```python
from build123d import *

# Parameters (mm, degrees)
BOSS_EXTRUDE1_DEPTH = 1440
SKETCH2_R           = 8.5
CUT_EXTRUDE1_DEPTH  = 1440


with BuildPart() as part:
    # Sketch1 → Boss-Extrude1 (new body)
    with BuildSketch(Plane.XY):
        with BuildLine():
            Line((0, 0), (-50, 0))
            Line((-50, 0), (-50, -100))
            Line((-50, -100), (0, -100))
            Line((0, -100), (0, -98.925311188))
            ThreePointArc((0, -98.925311188), (-1.103806889, -95.973045557), (-3.873721046, -94.469104878))
            Line((-3.873721046, -94.469104878), (-36.682971358, -89.858065454))
            ThreePointArc((-36.682971358, -89.858065454), (-41.915031432, -87.017288616), (-44, -81.440786869))
            Line((-44, -81.440786869), (-44, -18.559213131))
            ThreePointArc((-44, -18.559213131), (-41.915031432, -12.982711384), (-36.682971358, -10.141934546))
            Line((-36.682971358, -10.141934546), (-3.873721046, -5.530895122))
            ThreePointArc((-3.873721046, -5.530895122), (-1.103806889, -4.026954443), (0, -1.074688812))
            Line((0, -1.074688812), (0, 0))
        make_face()
    extrude(amount=BOSS_EXTRUDE1_DEPTH)

    # Sketch2 → Cut-Extrude1 (cut)
    with BuildSketch(Plane.ZY.offset(50)):
        with Locations(Location((73.2, -38, 0), (0, 0, 270))):
            Circle(SKETCH2_R)
        with Locations(Location((234.9, -38, 0), (0, 0, 270))):
            Circle(SKETCH2_R)
        with Locations(Location((396.6, -38, 0), (0, 0, 270))):
            Circle(SKETCH2_R)
        with Locations(Location((558.3, -38, 0), (0, 0, 270))):
            Circle(SKETCH2_R)
        with Locations(Location((720, -38, 0), (0, 0, 270))):
            Circle(SKETCH2_R)
        with Locations(Location((881.7, -38, 0), (0, 0, 270))):
            Circle(SKETCH2_R)
        with Locations(Location((1043.4, -38, 0), (0, 0, 270))):
            Circle(SKETCH2_R)
        with Locations(Location((1205.1, -38, 0), (0, 0, 270))):
            Circle(SKETCH2_R)
        with Locations(Location((1366.8, -38, 0), (0, 0, 270))):
            Circle(SKETCH2_R)
    extrude(amount=-CUT_EXTRUDE1_DEPTH, mode=Mode.SUBTRACT)


solid = part.part
```
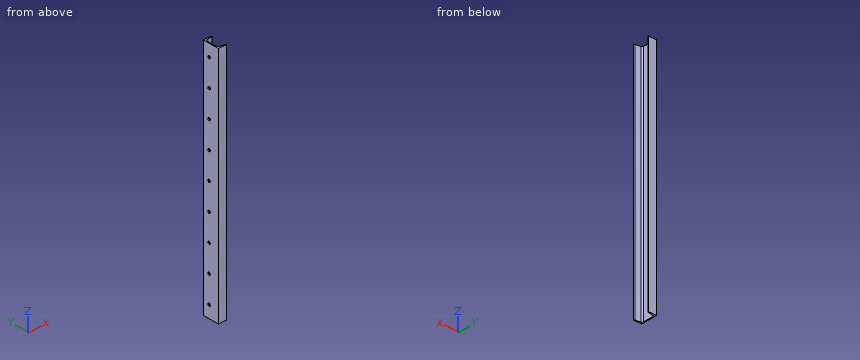
Work out the finished part from the listing and answer in its coordinate system (mm). Round coordinates to 2 decimals unless told otherwise and drop trailing zeros. Write each loop counter-clockwise with the first axis right and the second up, starting at its lowest first coordinate (ties: lowest second). Pieces come first, ordered by that corner, then holes.
1) A cutting plane is placed at A-A on x = -26. Determine the outline of the cut face in (y, z), and give its area (3 significant figures).
2) Consider probe 1 along Y at (x, z) = (-46, 396); probe 2 along Y at (x, z) = (-4, 325.5); probe 3 along X at (y, z) = (-51.5, 1370.5). Determine where each line is inside the solid, lowest interval first.
3) A cutting plane is placed at B-B on z = 685. Determine the outline of the cut face in (x, y), and give its area (3 significant figures).
4) Flat-ended cylindrical pins translate along their axes: P1, Ø3, axis at y = -85.5, z = 899.5, coming from the +X side; P2, Ø15.5, axis at y = -38, z = 881.7, coming from the -X side; P3, Ø8, axis at y = -20.5, z = 1242, coming from the +X side; P4, Ø8, axis at y = -70, z = 709, coming from the +X side. Find the tip coordinate at first contact, or state that the pin passes through.
Entries:
1. outline: (-100, 0) - (-91.36, 0) - (-91.36, 1440) - (-100, 1440) - close; (-8.64, 0) - (0, 0) - (0, 1440) - (-8.64, 1440) - close
1. area: 24,900 mm2
2. probe 1: y = -100 to -46.48, -29.52 to 0
2. probe 2: y = -100 to -94.45, -5.55 to 0
2. probe 3: x = -50 to -44
3. outline: (-50, -100) - (0, -100) - (0, -98.93) arc R4.5 ccw to (-3.87, -94.47) - (-36.68, -89.86) arc R8.5 cw to (-44, -81.44) - (-44, -18.56) arc R8.5 cw to (-36.68, -10.14) - (-3.87, -5.53) arc R4.5 ccw to (0, -1.07) - (0, 0) - (-50, 0) - close
3. area: 1,330 mm2
4. P1: stops at x = -41.93
4. P2: passes through
4. P3: stops at x = -43.75
4. P4: stops at x = -44
